Input: dimensioned drawing with shaded views. Units: mm. Origin: part minimum x, y, z. Coordinates: 2 decimals unless noted, no trailing zeros. Order: outer loops, then holes, each group sorted by start corner. A loop starts at its lowest first (then second) coordinate and runs counter-clockwise, first axis right, second up. Notation, with made-up numbers: (60, 57) -> (89, 57) arc R22 ccw to (89, 72) -> close; hole circle Ø2 at (30.5, 19). An arc over 180 degrees is marked (long way). Write item = value, one per line. Start each with the question number.
Item 1: Section query B-B (y = 20). Output: boundary loops of the cut face in (x, z), then the cut area to 3 significant figures.
Item 2: Contact query for a flat-ended pin moving along its axis: pin 1 (5 mm diameter, centred on x = 253.5, z = 4.5, fed in from -Y). Output: stop coordinate, or through.
Item 3: Section query A-A (y = 559.5). Output: boundary loops of the cut face in (x, z).
Item 4: Section query C-C (x = 20). Output: boundary loops of the cut face in (y, z).
Item 5: Ray query, line 1 along Y through (x, z) = (380, 5.5); line 2 along X through (y, z) = (980, 4.5); line 3 along X through (y, z) = (432, 3.5). Return the intervals inside material, ascending. Write a range as [from, to].
Item 6: Section query D-D (z = 2.5). Output: boundary loops of the cut face in (x, y).
Item 7: Mould query, pull axis Z, two halves, no side actions, for the marked faces 1 and 2. Classes: released by +Z, released by -Z, zero draft, split by the parting line, or undercut.
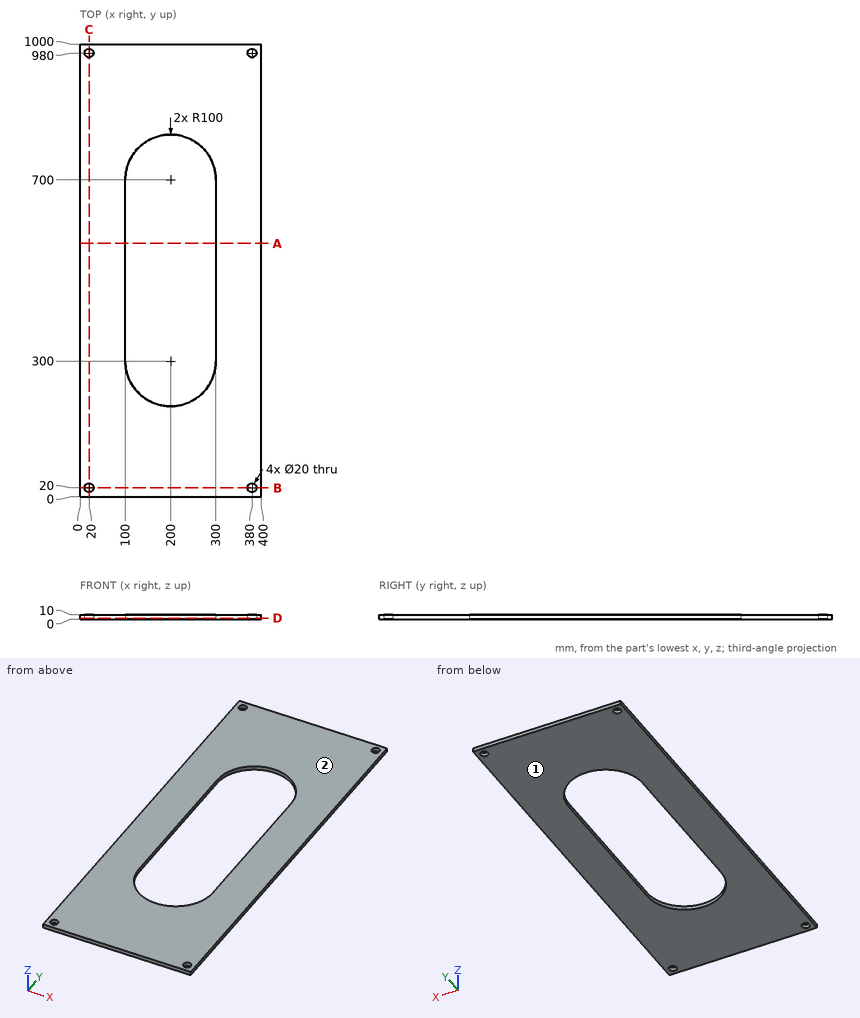
Computed:
q1.outline = (0, 0) -> (10, 0) -> (10, 10) -> (0, 10) -> close; (30, 0) -> (370, 0) -> (370, 10) -> (30, 10) -> close; (390, 0) -> (400, 0) -> (400, 10) -> (390, 10) -> close
q1.area = 3,600 mm^2
q2.pin_1 = 0
q3.outline = (0, 0) -> (100, 0) -> (100, 10) -> (0, 10) -> close; (300, 0) -> (400, 0) -> (400, 10) -> (300, 10) -> close
q4.outline = (0, 0) -> (10, 0) -> (10, 10) -> (0, 10) -> close; (30, 0) -> (970, 0) -> (970, 10) -> (30, 10) -> close; (990, 0) -> (1000, 0) -> (1000, 10) -> (990, 10) -> close
q5.line_1 = [0, 10], [30, 970], [990, 1000]
q5.line_2 = [0, 10], [30, 370], [390, 400]
q5.line_3 = [0, 100], [300, 400]
q6.outline = (0, 0) -> (400, 0) -> (400, 1000) -> (0, 1000) -> close; hole circle Ø20 at (20, 20); hole circle Ø20 at (20, 980); hole (100, 300) arc R100 ccw to (300, 300) -> (300, 700) arc R100 ccw to (100, 700) -> close; hole circle Ø20 at (380, 20); hole circle Ø20 at (380, 980)
q7.face_1 = released by -Z
q7.face_2 = released by +Z
